For this review, take the finished solid that the model builds, in its own axes (mm). Face numbers are marked on the shaded views. A direction names the side the tool comes from. Give positions to 0.01 mm unless a question says otherwise; leave off trailing zeros. Write each loop counter-clockwise with the first axis right and the second up, starting at its lowest first coordinate (ties: lowest second). Pieces come first, ordered by that corner, then holes.
Q1. We need section D-D (y = 7.5). Write out the cut boundary in (x, z), then the cut area to 3 significant figures.
Q2. Mouldability with a two-part tool opening along Z and no side actions: class the marked faces 1, 2 and 3 as released by +Z, released by -Z, zero draft, split by the parting line, or undercut.
Q3. We need section C-C (y = 54.5). Write out the cut boundary in (x, z), then the cut area to 3 significant figures.
Q4. Machinability: for the marked faces 4 and 5, which of the approach directions +Z, -Z, +X, -X, +Y, -Y give a long, thin tool a straight path to every point of the face, cutting with its end or side? Answer none if there is none.
Q5. For line 1 (X direction, y = 42, z = 0); line 2 (X direction, y = 56.5, z = 0); line 3 (Y direction, x = -11, z = -33.5), list the stretches that pass through material, from the lowest coordinate up.
Q6. We need section B-B (x = 0). Write out the cut boundary in (y, z), then the cut area to 3 significant figures.
Q7. We need section A-A (z = 0). Write out the cut boundary in (x, y), then the cut area to 3 significant figures.
Q8. Insertion check: P1, Ø1.5, axis at x = 35, z = -10, coming from the -Y side; P2, Ø4, axis at x = 5, z = 25.5, coming from the -Y side; P3, Ø4, axis at x = -9, y = 12.5, coming from the -Z side; P4, Ø1.5, axis at y = 30.5, z = -31, coming from the +X side. Each pin has a flat end and moves straight along its axis. Give the tip position at first contact, or say it passes through.
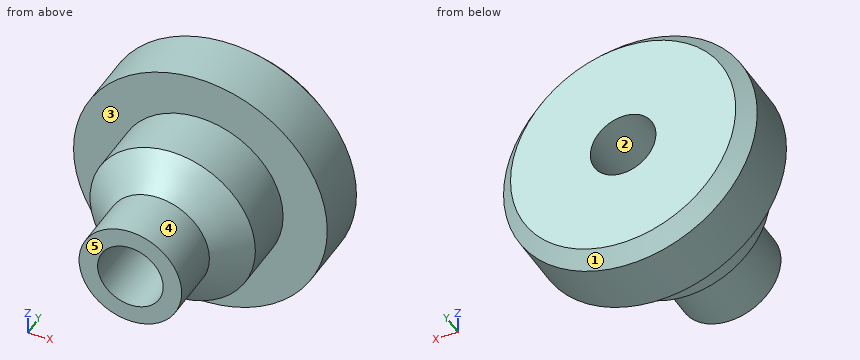
```python
from build123d import *

# Parameters (mm, degrees)
CHAMFER1_SIZE = 5


with BuildPart() as part:
    # Sketch1 → Revolve1 (revolve)
    with BuildSketch(Plane.XY):
        Polygon((11.5, 0), (11.5, 73), (44.5, 73), (44.5, 48), (29, 48), (29, 29), (18, 19), (18, 0), align=None)
    revolve(axis=Axis((0, -693.799212598, 0), (0, 1, 0)))

    # Chamfer1
    chamfer1_edges = [part.edges().sort_by_distance(p)[0] for p in [
        (-44.5, 73, 0),
    ]]
    chamfer(chamfer1_edges, length=CHAMFER1_SIZE)


solid = part.part
```
Computed:
1. outline: circle Ø36 at (0, 0); hole circle Ø23 at (0, 0)
1. area: 602 mm2
2. face 1: split by the parting line
2. face 2: undercut
2. face 3: zero draft
3. outline: circle Ø89 at (0, 0); hole circle Ø23 at (0, 0)
3. area: 5,810 mm2
4. face 4: -Y
4. face 5: +Z, -Z, +X, -X, -Y
5. line 1: x = -29 to -11.5, 11.5 to 29
5. line 2: x = -44.5 to -11.5, 11.5 to 44.5
5. line 3: y = 48 to 73
6. outline: (0, -18) - (19, -18) - (29, -29) - (48, -29) - (48, -44.5) - (68, -44.5) - (73, -39.5) - (73, -11.5) - (0, -11.5) - close; (0, 11.5) - (73, 11.5) - (73, 39.5) - (68, 44.5) - (48, 44.5) - (48, 29) - (29, 29) - (19, 18) - (0, 18) - close
6. area: 2,780 mm2
7. outline: (-44.5, 48) - (-29, 48) - (-29, 29) - (-18, 19) - (-18, 0) - (-11.5, 0) - (-11.5, 73) - (-39.5, 73) - (-44.5, 68) - close; (11.5, 0) - (18, 0) - (18, 19) - (29, 29) - (29, 48) - (44.5, 48) - (44.5, 68) - (39.5, 73) - (11.5, 73) - close
7. area: 2,780 mm2
8. P1: stops at y = 48
8. P2: stops at y = 24.44
8. P3: stops at z = -16.58
8. P4: passes through
